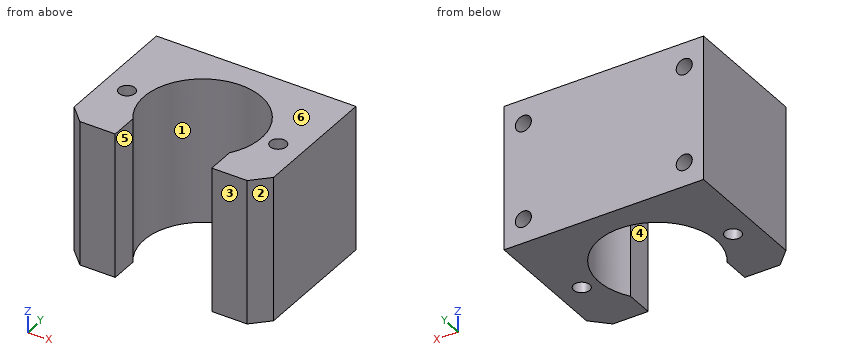
from build123d import *

# Parameters (mm, degrees)
SKETCH_1_W                  = 62
SKETCH_1_H                  = 45
EXTRUDE_1_DEPTH             = 22.5
CUT_EXTRUDE_1_DEPTH         = 45
CHAMFER_1_SIZE              = 5
HOLE_WIZARD_M6_1_D          = 5
HOLE_WIZARD_M6_1_DEPTH      = 15
HOLE_WIZARD_M6_1_TIP        = 1.502151548
HOLE_WIZARD_M6_2_AT_2_COUNT = 2
HOLE_WIZARD_M6_2_AT_2_PITCH = 47


with BuildPart() as part:
    # 草图1 → 凸台-拉伸1 (new, symmetric)
    with BuildSketch(Plane(origin=(0, 0, 0), x_dir=(1, 0, 0), z_dir=(0, 1, 0))):
        Rectangle(SKETCH_1_W, SKETCH_1_H)
    extrude(amount=EXTRUDE_1_DEPTH, both=True)

    # 草图2 → 切除-拉伸1 (cut)
    with BuildSketch(Plane(origin=(0, 0, -22.5), x_dir=(-1, 0, 0), z_dir=(0, 0, -1))):
        with BuildLine():
            Line((-15, -13.895311443), (-15, -22.5))
            Line((-15, -22.5), (15, -22.5))
            Line((15, -22.5), (15, -13.895311443))
            ThreePointArc((15, -13.895311443), (0, 14.75), (-15, -13.895311443))
        make_face()
    extrude(amount=-CUT_EXTRUDE_1_DEPTH, mode=Mode.SUBTRACT)

    # 倒角1
    chamfer_1_edges = [part.edges().sort_by_distance(p)[0] for p in [
        (-31, -22.5, 0),
        (31, -22.5, 0),
    ]]
    chamfer(chamfer_1_edges, length=CHAMFER_1_SIZE)

    # M6 螺纹孔1
    with Locations(Plane(origin=(0, 22.5, 0), x_dir=(1, 0, 0), z_dir=(0, 1, 0))):
        with Locations((-25, 15), (-25, -15), (25, -15), (25, 15)):
            Hole(HOLE_WIZARD_M6_1_D / 2, depth=HOLE_WIZARD_M6_1_DEPTH)
            with Locations((0, 0, -(HOLE_WIZARD_M6_1_DEPTH + HOLE_WIZARD_M6_1_TIP / 2))):  # 118° drill point
                Cone(0, HOLE_WIZARD_M6_1_D / 2, HOLE_WIZARD_M6_1_TIP, mode=Mode.SUBTRACT)

    # 草图6 → M6 螺纹孔2 (revolve, cut)
    with BuildSketch(Plane(origin=(23.5, -3.5, -22.5), x_dir=(0, 1, 0), z_dir=(1, 0, 0))):
        Polygon((0, 0), (0, 16.502151548), (2.5, 15), (2.5, 0), align=None)
    hole_wizard_m6_2 = revolve(axis=Axis((23.5, -3.5, -28.85), (0, 0, 1)), mode=Mode.SUBTRACT)

    # M6 螺纹孔2 at 2: M6 螺纹孔2 ×2
    with Locations(*[(-i * HOLE_WIZARD_M6_2_AT_2_PITCH, 0, 0) for i in range(1, HOLE_WIZARD_M6_2_AT_2_COUNT)]):
        add(hole_wizard_m6_2, mode=Mode.SUBTRACT)

    # 镜向1: M6 螺纹孔2 across plane
    add(hole_wizard_m6_2.mirror(Plane.XY), mode=Mode.SUBTRACT)

    # 镜向1 copy 1 sketch → 镜向1 copy 1 (revolve, cut)
    with BuildSketch(Plane(origin=(-23.5, -3.5, 22.5), x_dir=(0, 1, 0), z_dir=(1, 0, 0))):
        Polygon((0, 0), (0, -16.502151548), (2.5, -15), (2.5, 0), align=None)
    revolve(axis=Axis((-23.5, -3.5, 28.85), (0, 0, 1)), mode=Mode.SUBTRACT)


solid = part.part
Read the model definition and answer for the solid it produces. Units are mm, in the model's axes. Face numbers are marked on the shaded views. A direction names the side the tool comes from. Coordinates: 2 decimals unless noted, no trailing zeros. Order: outer loops, then holes, each group sorted by start corner. A loop starts at its lowest first (then second) coordinate and runs counter-clockwise, first axis right, second up. Notation, with made-up numbers: M 36,71.5 L 90,71.5 A7 cw 90,82.5 Z; hole C 60,86.25 d1. An arc over 180 degrees is marked long. Put each result on its own line as item: value. Start each with the question number.
Item 1: Consider probe 1 along X at (y, z) = (15, -15); probe 2 along Z at (x, y) = (-25, 14.5); probe 3 along X at (y, z) = (12, 15). Determine where each line is inside the solid, lowest interval first. Write a range as [from, to].
Item 2: Section C-C, the plane x = 0 is taken. Determine the outline of the cut face in (y, z).
Item 3: The mould has two halves that part along X. Classify the marked faces 1, 2, 3 and 4: +X half, -X half, draft (parallel to the pull), parting line (faces both ways), or undercut.
Item 4: For the marked faces 5 and 6, determine the directions among +Z, -Z, +X, -X, +Y, -Y from which every point of the face is accessible in a straight line to the end or side of a thin tool.
Item 5: Section B-B, the plane z = 16.5 is taken. Count the separate pieces of the cut face and the enclosed holes in it, plus the area to 3 significant figures.
Item 6: Section A-A, the plane y = -19 is taken. Determine the outline of the cut face in (x, z).
Item 7: Section D-D, the plane y = 0 is taken. Determine the outline of the cut face in (x, z).
Item 8: Given pin 1 Ø4 at (x, y) = (-23.5, -3.5) entering from -Z; pin 2 Ø1 at (x, z) = (8.5, -10.5) entering from -Y, each flat-ended and moving along its own axis, determine where each tip first touches the part or whether it passes through.
Computed:
1. probe 1: x = [-31, -27.5], [-22.5, 22.5], [27.5, 31]
1. probe 2: z = [-22.5, -17.5], [-12.5, 12.5], [17.5, 22.5]
1. probe 3: x = [-31, -27.5], [-22.5, -9.63], [9.63, 22.5], [27.5, 31]
2. outline: M 14.75,-22.5 L 22.5,-22.5 L 22.5,22.5 L 14.75,22.5 Z
3. face 1: undercut
3. face 2: +X half
3. face 3: draft
3. face 4: undercut
4. face 5: +Z, -Z, -Y
4. face 6: +Z, +X, -X, +Y, -Y
5. separate pieces: 1
5. enclosed holes: 2
5. area: 1,460 mm2
6. outline: M -29.5,-22.5 L -15,-22.5 L -15,22.5 L -29.5,22.5 Z; M 15,-22.5 L 29.5,-22.5 L 29.5,22.5 L 15,22.5 Z
7. outline: M -31,-22.5 L -17.91,-22.5 L -17.91,22.5 L -31,22.5 Z; M 17.91,-22.5 L 31,-22.5 L 31,22.5 L 17.91,22.5 Z
8. pin 1: stops at z = -7.2
8. pin 2: stops at y = 12.38
